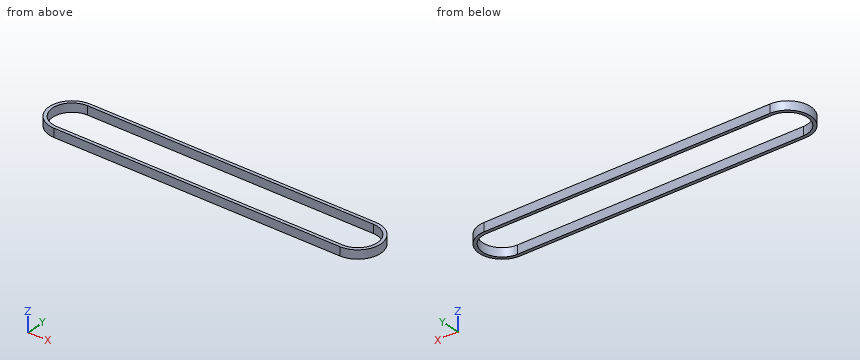
```python
from build123d import *

# Parameters (mm, degrees)
BOSS_EXTRUDE1_DEPTH = 7.9
SHELL1_T            = -3


with BuildPart() as part:
    # Sketch2 → Boss-Extrude1 (new body)
    with BuildSketch(Plane.XY):
        with BuildLine():
            Line((0, 20.9), (-260, 20.9))
            ThreePointArc((-260, 20.9), (-280.9, 0), (-260, -20.9))
            Line((-260, -20.9), (0, -20.9))
            ThreePointArc((0, -20.9), (20.9, 0), (0, 20.9))
        make_face()
    extrude(amount=BOSS_EXTRUDE1_DEPTH)

    # Shell1
    shell1_openings = [part.faces().sort_by_distance(p)[0] for p in [
        (-130, 0, 7.9),
        (-130, 0, 0),
    ]]
    offset(amount=SHELL1_T, openings=shell1_openings, kind=Kind.INTERSECTION)


solid = part.part
```
The listing builds one solid part. Answer for the finished solid, in the listing's coordinates (mm). Give positions to 0.01 mm unless a question says otherwise; leave off trailing zeros. Order: outer loops, then holes, each group sorted by start corner. A loop starts at its lowest first (then second) coordinate and runs counter-clockwise, first axis right, second up. Notation, with made-up numbers: (58.25, -37.75) -> (107.25, -37.75) arc R13 ccw to (107.25, -30.75) -> close; hole circle Ø9 at (89, 52). An arc over 180 degrees is marked (long way). Answer as CSV lines item,"result". Start each with the question number.
Q1. Find the intervals of material crossed by L1, parallel to Y at x = -224, z = 7.25; L2, parallel to X at y = 0, z = 2.5; L3, parallel to X at y = 14.5, z = 5.5, in increasing order.
Q2. A cutting plane is placed at A-A (y = 0). Determine the outline of the cut face in (x, z), then the cut area to 3 significant figures.
Q3. A cutting plane is placed at C-C (z = 6). Determine the outline of the cut face in (x, y), then the cut area to 3 significant figures.
Q4. A cutting plane is placed at B-B (x = -30). Determine the outline of the cut face in (y, z).
Q5. Given pin 1 (3 mm diameter, centred on y = -8, z = 6.5, fed in from -X); pin 2 (3 mm diameter, centred on y = 3.5, z = 2.5, fed in from -X), each flat-ended and moving along its own axis, determine where each tip first touches the part or whether it passes through.
Results found:
1,L1,"-20.9 to -17.9, 17.9 to 20.9"
1,L2,"-280.9 to -277.9, 17.9 to 20.9"
1,L3,"-275.05 to -270.5, 10.5 to 15.05"
2,outline,"(-280.9, 0) -> (-277.9, 0) -> (-277.9, 7.9) -> (-280.9, 7.9) -> close; (17.9, 0) -> (20.9, 0) -> (20.9, 7.9) -> (17.9, 7.9) -> close"
2,area,"47.4 mm2"
3,outline,"(-260, -20.9) -> (0, -20.9) arc R20.9 ccw to (0, 20.9) -> (-260, 20.9) arc R20.9 ccw to start; hole (-260, -17.9) -> (0, -17.9) arc R17.9 ccw to (0, 17.9) -> (-260, 17.9) arc R17.9 ccw to start"
3,area,"1,930 mm2"
4,outline,"(-20.9, 0) -> (-17.9, 0) -> (-17.9, 7.9) -> (-20.9, 7.9) -> close; (17.9, 0) -> (20.9, 0) -> (20.9, 7.9) -> (17.9, 7.9) -> close"
5,pin 1,"x = -279.86"
5,pin 2,"x = -280.8"
